The listing builds one solid part. Answer for the finished solid, in the listing's coordinates (mm). Round coordinates to 2 decimals unless told otherwise and drop trailing zeros. Loops run counter-clockwise (first coordinate to the right, second up) from the corner with the lowest first, then second, coordinate; pieces in that order, holes last. Notation, with made-up numbers: M 85.25,33 L 132.25,33 A16 ccw 132.25,53 Z; hole C 77,-21 d11. An arc over 180 degrees is marked long. Put each result on its own line as item: value. Start each with the question number.
(1) Straight lines are drawn through the part: line 1 (Y direction, x = -216.5, z = 1.75); line 2 (X direction, y = 198, z = 3.75) (3 decimals); line 3 (X direction, y = 134, z = -1.25) (3 decimals). For each, find the intervals that lie inside material, in ascending order.
(2) Section C-C, the plane y = 118.5 is taken. Determine the outline of the cut face in (x, z).
(3) Section B-B, the plane z = -3.75 is taken. Determine the outline of the cut face in (x, y) (3 decimals), then the cut area to 3 significant figures.
(4) Flat-ended cylindrical pins translate along their axes: P1, Ø6, axis at x = -88, z = -2, coming from the +Y side; P2, Ø3.5, axis at y = 116.5, z = -2.5, coming from the +X side. Find the tip coordinate at first contact, or state that the pin passes through.
(5) Section A-A, the plane x = -193 is taken. Determine the outline of the cut face in (y, z).
(6) Section D-D, the plane x = -16.5 is taken. Determine the outline of the cut face in (y, z).
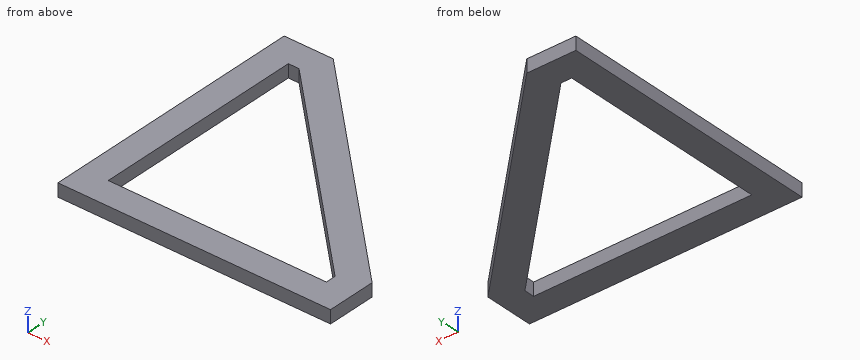
```python
from build123d import *

# Parameters (mm, degrees)
EXTRUDE_1_DEPTH = 6


with BuildPart() as part:
    # 草图1 → 凸台-拉伸1 (new, symmetric)
    with BuildSketch(Plane.XY):
        Polygon((0, 0), (-250, 0), (-250, 245), (-205, 245), (0, 45), align=None)
        Polygon((-225, 220), (-215.175008729, 220), (-25, 34.463406118), (-25, 25), (-225, 25), align=None, mode=Mode.SUBTRACT)
    extrude(amount=EXTRUDE_1_DEPTH, both=True)


solid = part.part
```
Recorded:
1. line 1: y = 0 to 25, 220 to 245
1. line 2: x = -250 to -225, -192.625 to -156.825
1. line 3: x = -250 to -225, -127.025 to -91.225
2. outline: M -250,-6 L -225,-6 L -225,6 L -250,6 Z; M -111.14,-6 L -75.34,-6 L -75.34,6 L -111.14,6 Z
3. outline: M -250,0 L 0,0 L 0,45 L -205,245 L -250,245 Z; hole M -225,25 L -25,25 L -25,34.463 L -215.175,220 L -225,220 Z
3. area: 19,400 mm²
4. P1: stops at y = 133.78
4. P2: stops at x = -71.49
5. outline: M 0,-6 L 25,-6 L 25,6 L 0,6 Z; M 198.37,-6 L 233.29,-6 L 233.29,6 L 198.37,6 Z
6. outline: M 0,-6 L 61.1,-6 L 61.1,6 L 0,6 Z
